Work out the finished part from the listing and answer in its coordinate system (mm). Face numbers are marked on the shaded views. Coordinates: 2 decimals unless noted, no trailing zeros. Write each loop counter-clockwise with the first axis right and the second up, starting at its lowest first coordinate (ties: lowest second). Pieces come first, ordered by that corner, then holes. Notation, with made-up numbers: (53, 55) - (58, 55) arc R14 cw to (58, 79) - close; hole circle Ø6 at (85, -12.5). An arc over 180 degrees is marked (long way). Answer as a JSON object with one key per item and string values. Group by question number.
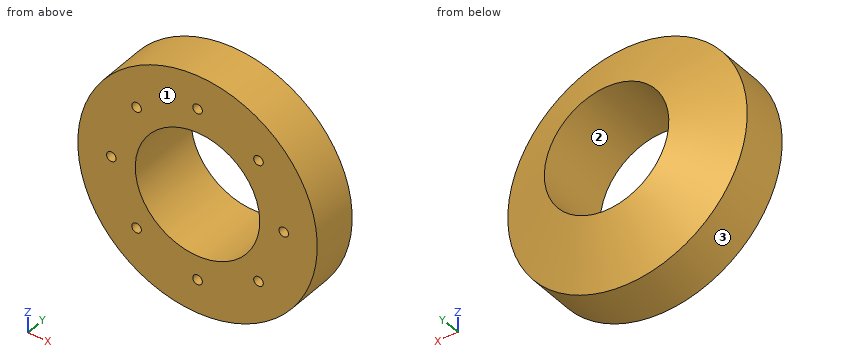
from build123d import *

# Parameters (mm, degrees)
SKETCH_2_R          = 5
CUT_EXTRUDE_1_DEPTH = 30


with BuildPart() as part:
    # 草图1 → 旋转1 (revolve)
    with BuildSketch(Plane.XY, mode=Mode.PRIVATE) as revolve_1_sk:
        Polygon((65, -53.991935484), (65, 26.008064516), (125, -3.991935484), (125, -53.991935484), align=None)
    revolve(revolve_1_sk.sketch.rotate(Axis((0, 116.89516129, 0), (0, -1, 0)), 90), axis=Axis((0, 116.89516129, 0), (0, -1, 0)))

    # 草图2 → 切除-拉伸1 (cut)
    with BuildSketch(Plane.XZ.offset(53.991935484)):
        with Locations(Location((90, 0, 0), (0, 0, 270))):
            Circle(SKETCH_2_R)
        with Locations(Location((63.639610307, -63.639610307, 0), (0, 0, 270))):
            Circle(SKETCH_2_R)
        with Locations(Location((0, -90, 0), (0, 0, 270))):
            Circle(SKETCH_2_R)
        with Locations(Location((-63.639610307, -63.639610307, 0), (0, 0, 270))):
            Circle(SKETCH_2_R)
        with Locations(Location((-90, 0, 0), (0, 0, 270))):
            Circle(SKETCH_2_R)
        with Locations(Location((-63.639610307, 63.639610307, 0), (0, 0, 270))):
            Circle(SKETCH_2_R)
        with Locations(Location((0, 90, 0), (0, 0, 270))):
            Circle(SKETCH_2_R)
        with Locations(Location((63.639610307, 63.639610307, 0), (0, 0, 270))):
            Circle(SKETCH_2_R)
    extrude(amount=-CUT_EXTRUDE_1_DEPTH, mode=Mode.SUBTRACT)


solid = part.part
Q1. Flat-ended cylindrical pins translate along their axes: pin 1 Ø12 at (y, z) = (-45, 14) entering from +X; pin 2 Ø11.5 at (x, z) = (-90, 0) entering from +Y; pin 3 Ø1 at (x, y) = (80.5, -22) entering from +Z. Find the tip coordinate at first contact, or state that the pin passes through.
Q2. Section B-B on z = 0 is taken. Determine the outline of the cut face in (x, y), plus the area to 3 significant figures.
Q3. Section C-C on y = -14 is taken. Determine the outline of the cut face in (x, z), plus the area to 3 significant figures.
Q4. Section A-A on x = 0 is taken. Determine the outline of the cut face in (y, z), plus the area to 3 significant figures.
Q5. Consider L1, parallel to X at y = -37.5, z = 0; L2, parallel to X at y = -27.5, z = -68; L3, parallel to Z at x = -36, y = -15.5. Determine where each line is inside the solid, lowest interval first. Write a range as from..to.
Q6. For a pull along X with two mould halves and no side action, classify the marked faces 1, 2 and 3 as +X half, -X half, draft (parallel to the pull), parting line (faces both ways), or undercut.
Q7. Section D-D on y = -31.5 is taken. Count the separate pieces of the cut face and the enclosed holes in it, plus the area to 3 significant figures.
Numbers:
{
 "1": {"pin 1": "stops at x = 124.74", "pin 2": "stops at y = 16.38", "pin 3": "stops at z = 96.05"},
 "2": {"outline": "(-125, -53.99) - (-95, -53.99) - (-95, -23.99) - (-85, -23.99) - (-85, -53.99) - (-65, -53.99) - (-65, 26.01) - (-125, -3.99) - close; (65, -53.99) - (85, -53.99) - (85, -23.99) - (95, -23.99) - (95, -53.99) - (125, -53.99) - (125, -3.99) - (65, 26.01) - close", "area": "7,200 mm²"},
 "3": {"outline": "circle Ø250 at (0, 0); hole circle Ø130 at (0, 0)", "area": "35,800 mm²"},
 "4": {"outline": "(-53.99, -125) - (-3.99, -125) - (26.01, -65) - (-53.99, -65) - (-53.99, -85) - (-23.99, -85) - (-23.99, -95) - (-53.99, -95) - close; (-53.99, 65) - (26.01, 65) - (-3.99, 125) - (-53.99, 125) - (-53.99, 95) - (-23.99, 95) - (-23.99, 85) - (-53.99, 85) - close", "area": "7,200 mm²"},
 "5": {"L1": "x = -125..-95, -85..-65, 65..85, 95..125", "L2": "x = -104.89..-66.09, -61.19..61.19, 66.09..104.89", "L3": "z = -119.7..-54.12, 54.12..119.7"},
 "6": {"face 1": "draft", "face 2": "undercut", "face 3": "parting line"},
 "7": {"separate pieces": "1", "enclosed holes": "9", "area": "35,200 mm²"}
}
